from build123d import *

# Parameters (mm, degrees)
BASE_PLATE_DEPTH            = 45
MOUNTING_HOLES_SKETCH_R     = 6
MOUNTING_HOLES_DEPTH        = 40
PIVOT_BOSS_PROFILE_R        = 10
PIVOT_BOSS_DEPTH            = 75
CENTER_GUSSET_RIB_REACH     = 119.5
CENTER_GUSSET_SKETCH_WALL_W = 317.777472108
CENTER_GUSSET_SKETCH_WALL_H = 10
SIDE_GUSSET_RIB_REACH       = 119.5
SIDE_GUSSET_SKETCH_WALL_W   = 268.622776602
SIDE_GUSSET_SKETCH_WALL_H   = 10


with BuildPart() as part:
    # Base Plate Profile → Base Plate (new, symmetric)
    with BuildSketch(Plane.XY):
        Polygon((-67.5, 0), (-27.5, 0), (-27.5, 10), (27.5, 10), (27.5, 0), (67.5, 0), (67.5, 10), (37.5, 10), (37.5, 20), (-37.5, 20), (-37.5, 10), (-67.5, 10), align=None)
    extrude(amount=BASE_PLATE_DEPTH, both=True)

    # Mounting Holes Sketch → Mounting Holes (cut)
    with BuildSketch(Plane(origin=(0, 10, 0), x_dir=(1, 0, 0), z_dir=(0, 1, 0))):
        with Locations(Location((52.5, -25, 0), (0, 0, 180))):
            Circle(MOUNTING_HOLES_SKETCH_R)
        with Locations(Location((52.5, 25, 0), (0, 0, 180))):
            Circle(MOUNTING_HOLES_SKETCH_R)
        with Locations(Location((-52.5, 25, 0), (0, 0, 270))):
            Circle(MOUNTING_HOLES_SKETCH_R)
        with Locations(Location((-52.5, -25, 0), (0, 0, 270))):
            Circle(MOUNTING_HOLES_SKETCH_R)
    extrude(amount=-MOUNTING_HOLES_DEPTH, mode=Mode.SUBTRACT)

    # Pivot Boss Profile → Pivot Boss (add)
    with BuildSketch(Plane(origin=(37.5, 0, 0), x_dir=(0, 0, -1), z_dir=(1, 0, 0))):
        with BuildLine():
            Line((45, 20), (5, 20))
            Line((5, 20), (5, 65))
            ThreePointArc((5, 65), (25, 85), (45, 65))
            Line((45, 65), (45, 20))
        make_face()
        with Locations((25, 65)):
            Circle(PIVOT_BOSS_PROFILE_R, mode=Mode.SUBTRACT)
    extrude(amount=-PIVOT_BOSS_DEPTH)

    # Center Gusset Sketch wall → Center Gusset Rib (add, up to next)
    with BuildSketch(Plane(origin=(0, 49.365592849, 17.270738259), x_dir=(0, -0.727073825966, 0.686559284837), z_dir=(0, -0.686559284837, -0.727073825966)), mode=Mode.PRIVATE) as center_gusset_rib_sk1:
        Rectangle(CENTER_GUSSET_SKETCH_WALL_W, CENTER_GUSSET_SKETCH_WALL_H)
    center_gusset_rib_tool1 = extrude(center_gusset_rib_sk1.sketch, amount=CENTER_GUSSET_RIB_REACH, mode=Mode.PRIVATE) - part.part
    add(center_gusset_rib_tool1.solids().sort_by_distance((0, 49.365592849, 17.270738259))[0])

    # Side Gusset Sketch wall → Side Gusset Rib (add, up to next)
    with BuildSketch(Plane(origin=(-52.5, 15, 0), x_dir=(-0.948683298051, -0.316227766017, 0), z_dir=(0.316227766017, -0.948683298051, 0)), mode=Mode.PRIVATE) as side_gusset_rib_sk1:
        Rectangle(SIDE_GUSSET_SKETCH_WALL_W, SIDE_GUSSET_SKETCH_WALL_H)
    side_gusset_rib_tool1 = extrude(side_gusset_rib_sk1.sketch, amount=SIDE_GUSSET_RIB_REACH, mode=Mode.PRIVATE) - part.part
    side_gusset_rib = side_gusset_rib_tool1.solids().sort_by_distance((-52.5, 15, 0))[0]
    add(side_gusset_rib)

    # Side Gusset Mirror: Side Gusset Rib across plane
    add(side_gusset_rib.mirror(Plane(origin=(0, 0, 0), x_dir=(0, 0, 1), z_dir=(1, 0, 0))))


solid = part.part
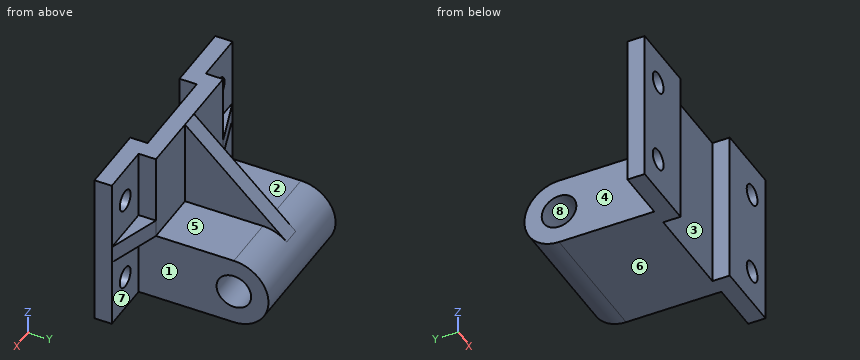
Can you work these out from the model? Positions are in its coordinate system, mm. Face numbers are marked on the shaded views. A direction names the side the tool comes from. Coordinates: 2 decimals unless noted, no trailing zeros. Loops run counter-clockwise (first coordinate to the right, second up) from the corner with the lowest first, then second, coordinate; pieces in that order, holes last. Notation, with made-up numbers: M 40.5,6 L 84.5,6 A14 cw 84.5,20 Z; hole C 60,29.25 d9. An arc over 180 degrees is marked long. Return JSON: item names as keys, results as strings. Group by question number.
Item 1: Imagine slicing it at C-C (x = 30). Please give me the cut outline in (y, z), and give its area (3 significant figures).
Item 2: Imagine slicing it at D-D (z = 25). Please give me the cut outline in (x, y), and give its area (3 significant figures).
Item 3: Thinking about a two-plate mould opening in Z: for the marked faces 6, 7 and 8, which applies, released by +Z, released by -Z, zero draft, split by the parting line, or undercut?
Item 4: I'm going to push flat-ended pins straight in: pin 1 Ø11 at (x, y) = (-54.5, 16.5) entering from +Z; pin 2 Ø5 at (y, z) = (29.5, -19) entering from -X; pin 3 Ø11 at (y, z) = (16, 27) entering from +X. Where does each tip first touch, or does it pass through?
Item 5: Imagine slicing it at A-A (x = -52.5). Please give me the cut outline in (y, z).
Item 6: If I drill on L1, parallel to Z at x = 52, y = 3; L2, parallel to Z at x = -54, y = 9; L3, parallel to Y at x = -45, z = 9.5, over which ranges is the centre line in solid material (lowest first)? Write a range as from..to.
Item 7: Imagine slicing it at B-B (z = -25). Please give me the cut outline in (x, y).
Item 8: On a 3-axis mill with a long thin cutter (end or side, diameter ignored), from which of +Z, -Z, +X, -X, +Y, -Y can I reach the whole of each face in a straight line? I mean the marked faces 1, 2, 3, 4 and 5. Say none if no direction works.
Verdict:
{
 "1": {"outline": "M 0,-45 L 65,-45 A20 ccw 65,-5 L 20,-5 L 20,45 L 0,45 Z; hole C 65,-25 d20", "area": "3,910 mm^2"},
 "2": {"outline": "M -67.5,0 L -58.5,0 L -58.5,10 L -67.5,10 Z; M -46.5,0 L -27.5,0 L -27.5,10 L 27.5,10 L 27.5,0 L 46.5,0 L 46.5,10 L 37.5,10 L 37.5,20 L 5,20 L 5,41.18 L -5,41.18 L -5,20 L -37.5,20 L -37.5,10 L -46.5,10 Z; M 58.5,0 L 67.5,0 L 67.5,10 L 58.5,10 Z", "area": "1,520 mm^2"},
 "3": {"face 6": "released by -Z", "face 7": "zero draft", "face 8": "undercut"},
 "4": {"pin 1": "stops at z = 5", "pin 2": "stops at x = -37.5", "pin 3": "stops at x = 37.5"},
 "5": {"outline": "M 0,-45 L 10,-45 L 10,-31 L 0,-31 Z; M 0,-19 L 10,-19 L 10,-5 L 15,-5 L 15,5 L 10,5 L 10,19 L 0,19 Z; M 0,31 L 10,31 L 10,45 L 0,45 Z"},
 "6": {"L1": "z = -45..-30.98, -19.02..19.02, 30.98..45", "L2": "z = -45..-30.81, -19.19..19.19, 30.81..45", "L3": "y = 0..10"},
 "7": {"outline": "M -67.5,0 L -58.5,0 L -58.5,10 L -67.5,10 Z; M -46.5,0 L -27.5,0 L -27.5,10 L 27.5,10 L 27.5,0 L 46.5,0 L 46.5,10 L 37.5,10 L 37.5,55 L -37.5,55 L -37.5,10 L -46.5,10 Z; M -37.5,75 L 37.5,75 L 37.5,85 L -37.5,85 Z; M 58.5,0 L 67.5,0 L 67.5,10 L 58.5,10 Z"},
 "8": {"face 1": "-Z, +X, +Y", "face 2": "+Z, -X, +Y", "face 3": "+Z, -Z, -Y", "face 4": "-Z, -X, +Y", "face 5": "+Z, +X, +Y"}
}
